Part print with two shaded views. Sizes in mm from the minimum x, y, z corner. A direction names the side the tool comes from. Give positions to 0.01 mm unless a question says otherwise; leave off trailing zeros. Write each loop counter-clockwise with the first axis right and the second up, starting at its lowest first coordinate (ties: lowest second). Pieces come first, ordered by that corner, then holes. Notation, with made-up numbers: (-3, 15.25) -> (17, 15.25) arc R19 ccw to (17, 31.25) -> close; hole circle Ø3 at (71, -30). An arc over 180 degrees is marked (long way). Answer as a JSON object with one key per item and string values.
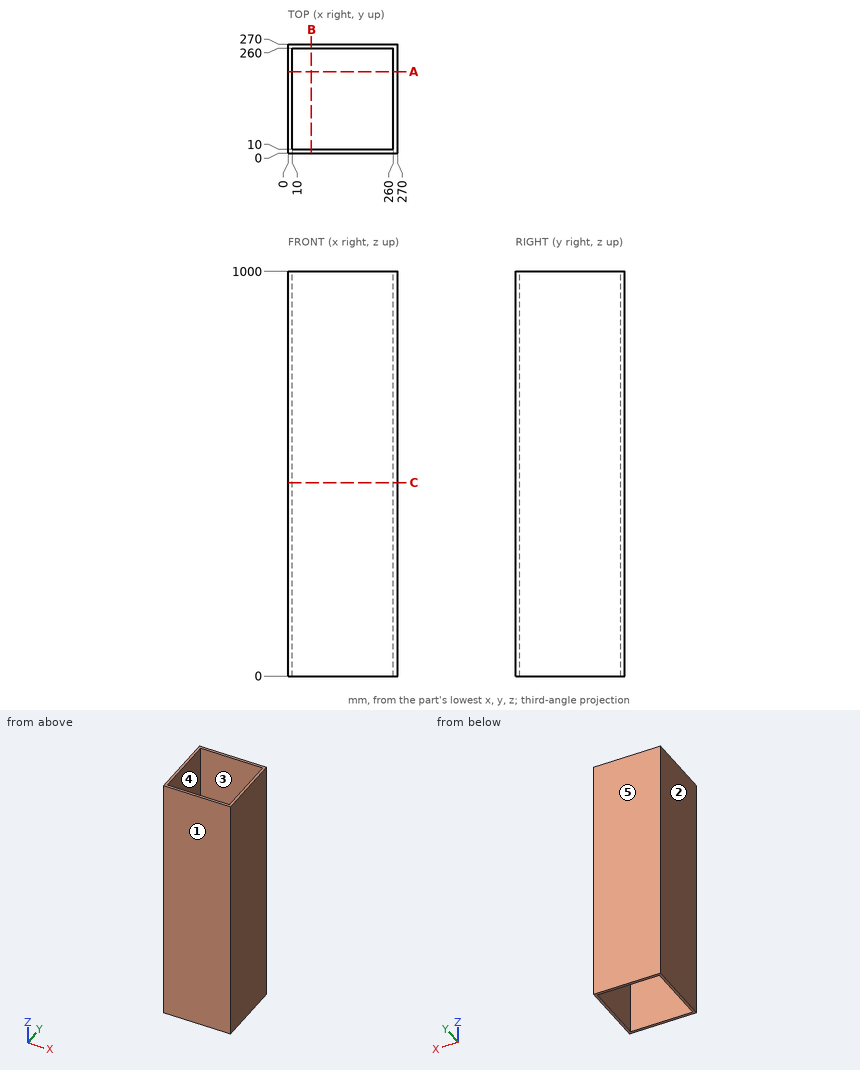
1) 3-axis set-ups, long thin cutter, end or side, ignore diameter. For the marked faces 4 and 5: which of +Z, -Z, +X, -X, +Y, -Y reach the whole face in a straight line?
Model answer:
{"face 4": "+Z, -Z", "face 5": "+Z, -Z, +X, -X, +Y"}
2) Slice it at C-C (z = 478). List the corners of the cut face in (x, y).
Model answer:
{"outline": "(0, 0) -> (270, 0) -> (270, 270) -> (0, 270) -> close; hole (10, 10) -> (260, 10) -> (260, 260) -> (10, 260) -> close"}
3) Wall check: probe 1 along Y at (x, z) = (138.5, 159). Give the ranges that are in metal, low to high.
Model answer:
{"probe 1": "y = 0 to 10, 260 to 270"}
4) Slice it at A-A (y = 202). List the corners of the cut face in (x, z), then the cut area to 3 significant figures.
Model answer:
{"outline": "(0, 0) -> (10, 0) -> (10, 1000) -> (0, 1000) -> close; (260, 0) -> (270, 0) -> (270, 1000) -> (260, 1000) -> close", "area": "20,000 mm2"}
5) Mould opens along Y. For the marked faces 1, 2 and 3 say: released by +Y, released by -Y, zero draft, split by the parting line, or undercut.
Model answer:
{"face 1": "released by -Y", "face 2": "zero draft", "face 3": "undercut"}
